Could you check a few things on this model? Use its own coordinates, in mm. A direction names the side the tool comes from. Round coordinates to 2 decimals unless told otherwise and drop trailing zeros. Write each loop counter-clockwise with the first axis right and the second up, starting at its lowest first coordinate (ties: lowest second). Pieces come first, ordered by that corner, then holes. Notation, with made-up numbers: (86, -28) - (133, -28) arc R9 cw to (133, -15) - close; hole circle Ø9 at (-36.75, 67.25). An arc over 180 degrees is marked (long way). Write each question's results on one line, items separated by ' | '. Start each with the question number.
(1) Imagine slicing it at A-A on x = 0. Write out the boundary of the cut face in (y, z).
(2) Please list where these lines run through material, in increasing order: line 1 (X direction, y = 0.75, z = 183); line 2 (Z direction, x = -3, y = 3.5); line 3 (Z direction, x = 3.5, y = -5). Write a range as [from, to].
(3) Imagine slicing it at C-C on z = 103.5. Write out the boundary of the cut face in (x, y).
(4) On a 3-axis mill with a long thin cutter (end or side, diameter ignored), from which of +Z, -Z, +X, -X, +Y, -Y can I reach the whole of each face in a straight line? I mean faces 1 (the flat face through (0, 0, 0)), 2 (the cylindrical face through (-6, 0, 15)), 3 (the cylindrical face through (-0.59, 4.46, 315.45)). Say none if no direction works.
(5) For P1, Ø1, axis at x = -2, z = 156, coming from the -Y side; P2, Ø6, axis at x = 0.5, z = 35, coming from the -Y side; P3, Ø3, axis at x = 5.5, y = -3.5, coming from the +Z side; P4, Ø2, axis at x = -4.5, z = 177.5, coming from the -Y side, each with a flat end and sliding along its axis, tell me the tip position at first contact or that it passes through.
```python
from build123d import *

# Parameters (mm, degrees)
SKETCH_1_R      = 4.5
EXTRUDE_1_DEPTH = 8
SKETCH_2_R      = 6
EXTRUDE_2_DEPTH = 14
SKETCH_3_R      = 7.5
EXTRUDE_3_DEPTH = 276
SKETCH_4_R      = 6
EXTRUDE_4_DEPTH = 14
SKETCH_5_R      = 4.5
EXTRUDE_5_DEPTH = 8
CHAMFER_1_SIZE  = 1


with BuildPart() as part:
    # 草图1 → 凸台-拉伸1 (new body)
    with BuildSketch(Plane.XY):
        Circle(SKETCH_1_R)
    extrude(amount=EXTRUDE_1_DEPTH)

    # 草图2 → 凸台-拉伸2 (add)
    with BuildSketch(Plane.XY.offset(8)):
        Circle(SKETCH_2_R)
    extrude(amount=EXTRUDE_2_DEPTH)

    # 草图3 → 凸台-拉伸3 (add)
    with BuildSketch(Plane.XY.offset(22)):
        Circle(SKETCH_3_R)
    extrude(amount=EXTRUDE_3_DEPTH)

    # 草图4 → 凸台-拉伸4 (add)
    with BuildSketch(Plane.XY.offset(298)):
        Circle(SKETCH_4_R)
    extrude(amount=EXTRUDE_4_DEPTH)

    # 草图5 → 凸台-拉伸5 (add)
    with BuildSketch(Plane.XY.offset(312)):
        Circle(SKETCH_5_R)
    extrude(amount=EXTRUDE_5_DEPTH)

    # 倒角1
    chamfer_1_edges = [part.edges().sort_by_distance(p)[0] for p in [
        (-4.5, 0, 0),
        (-4.5, 0, 320),
    ]]
    chamfer(chamfer_1_edges, length=CHAMFER_1_SIZE)


solid = part.part
```
Response:
1) outline: (-7.5, 22) - (-6, 22) - (-6, 8) - (-4.5, 8) - (-4.5, 1) - (-3.5, 0) - (3.5, 0) - (4.5, 1) - (4.5, 8) - (6, 8) - (6, 22) - (7.5, 22) - (7.5, 298) - (6, 298) - (6, 312) - (4.5, 312) - (4.5, 319) - (3.5, 320) - (-3.5, 320) - (-4.5, 319) - (-4.5, 312) - (-6, 312) - (-6, 298) - (-7.5, 298) - close
2) line 1: [-7.46, 7.46] | line 2: [8, 312] | line 3: [22, 298]
3) outline: circle Ø15 at (0, 0)
4) face 1: -Z, +X, -X, +Y, -Y | face 2: -Z | face 3: +Z
5) P1: y = -7.35 | P2: y = -7.5 | P3: z = 312 | P4: y = -6.63
